Here's how the part is built. I have some questions about the finished solid (model axes, mm). A direction names the side the tool comes from. Give positions to 0.01 mm unless a question says otherwise; leave off trailing zeros. Loops run counter-clockwise (first coordinate to the right, second up) from the corner with the lowest first, then second, coordinate; pieces in that order, holes last. Notation, with made-up numbers: (70.5, 6.25) - (92.5, 6.25) arc R14 cw to (92.5, 24.25) - close; hole circle Ø8 at (-32, 35.25). An arc over 180 degrees is marked (long way). Use a Markdown table: item, result.
from build123d import *

# Parameters (mm, degrees)
SKETCH_1_W             = 43
SKETCH_1_H             = 44
EXTRUDE_1_DEPTH        = 17.5
SKETCH_2_W             = 50
SKETCH_2_H             = 68
CUT_EXTRUDE_1_DEPTH    = 52.373631369
HOLE_WIZARD_M4_1_D     = 3.3
HOLE_WIZARD_M4_1_DEPTH = 15.5
HOLE_WIZARD_M4_1_TIP   = 0.991420021
CHAMFER_1_SIZE         = 5
HOLE_WIZARD_M4_2_D     = 3.3
HOLE_WIZARD_M4_2_DEPTH = 15.5
HOLE_WIZARD_M4_2_TIP   = 0.991420021


with BuildPart() as part:
    # 草图1 → 凸台-拉伸1 (new, symmetric)
    with BuildSketch(Plane.XY):
        Rectangle(SKETCH_1_W, SKETCH_1_H)
    extrude(amount=EXTRUDE_1_DEPTH, both=True)

    # 草图2 → 切除-拉伸1 (cut, through all)
    with BuildSketch(Plane(origin=(21.5, 0, 0), x_dir=(0, 0, -1), z_dir=(1, 0, 0))):
        with Locations((17.5, -22)):
            Rectangle(SKETCH_2_W, SKETCH_2_H)
    extrude(amount=-CUT_EXTRUDE_1_DEPTH, mode=Mode.SUBTRACT)

    # M4 螺纹孔1
    with Locations(Plane(origin=(0, 0, -17.5), x_dir=(-1, 0, 0), z_dir=(0, 0, -1))):
        with Locations((-15, 17), (15, 17)):
            Hole(HOLE_WIZARD_M4_1_D / 2, depth=HOLE_WIZARD_M4_1_DEPTH)
            with Locations((0, 0, -(HOLE_WIZARD_M4_1_DEPTH + HOLE_WIZARD_M4_1_TIP / 2))):  # 118° drill point
                Cone(0, HOLE_WIZARD_M4_1_D / 2, HOLE_WIZARD_M4_1_TIP, mode=Mode.SUBTRACT)

    # 倒角1
    chamfer_1_edges = [part.edges().sort_by_distance(p)[0] for p in [
        (0, 22, 17.5),
    ]]
    chamfer(chamfer_1_edges, length=CHAMFER_1_SIZE)

    # M4 螺纹孔2
    with Locations(Plane(origin=(0, -22, 0), x_dir=(-1, 0, 0), z_dir=(0, -1, 0))):
        with Locations((10, -12.5), (-10, -12.5)):
            Hole(HOLE_WIZARD_M4_2_D / 2, depth=HOLE_WIZARD_M4_2_DEPTH)
            with Locations((0, 0, -(HOLE_WIZARD_M4_2_DEPTH + HOLE_WIZARD_M4_2_TIP / 2))):  # 118° drill point
                Cone(0, HOLE_WIZARD_M4_2_D / 2, HOLE_WIZARD_M4_2_TIP, mode=Mode.SUBTRACT)


solid = part.part
(1) Suppose I cut it at A-A on x = -19. Write out the boundary of the cut face in (y, z).
A:
| item | result |
|---|---|
| outline | (-22, 7.5) - (12, 7.5) - (12, -17.5) - (22, -17.5) - (22, 12.5) - (17, 17.5) - (-22, 17.5) - close |
(2) On a 3-axis mill with a long thin cutter (end or side, diameter ignored), from which of +Z, -Z, +X, -X, +Y, -Y can I reach the whole of each face in a straight line? I mean faces 4 (the face through (16.574, 17.496, -9.642)), 5 (the face through (21.5, 5, 8)), 6 (the face through (10.761, -14.142, 13.964)), 7 (the face through (0, 12, -5)). Say none if no direction works.
A:
| item | result |
|---|---|
| face 4 | -Z |
| face 5 | +Z, -Z, +X, +Y, -Y |
| face 6 | -Y |
| face 7 | -Z, +X, -X, -Y |
(3) Suppose I cut it at B-B on y = -11. Write out the boundary of the cut face in (x, z).
A:
| item | result |
|---|---|
| outline | (-21.5, 7.5) - (21.5, 7.5) - (21.5, 17.5) - (-21.5, 17.5) - close; hole circle Ø3.3 at (-10, 12.5); hole circle Ø3.3 at (10, 12.5) |
(4) If I drill on line 1 (X direction, y = 17, z = -5.5); line 2 (X direction, y = -10.25, z = 12.5); line 3 (Z direction, x = 10, y = -9.75), over which ranges is the centre line in solid material (lowest first)?
A:
| item | result |
|---|---|
| line 1 | -21.5 to -16.65, -13.35 to 13.35, 16.65 to 21.5 |
| line 2 | -21.5 to -11.65, -8.35 to 8.35, 11.65 to 21.5 |
| line 3 | 7.5 to 10.85, 14.15 to 17.5 |
(5) Suppose I cut it at C-C on y = -1.5. Write out the boundary of the cut face in (x, z).
A:
| item | result |
|---|---|
| outline | (-21.5, 7.5) - (21.5, 7.5) - (21.5, 17.5) - (-21.5, 17.5) - close |
(6) We'd pull the mould along X, two halves only. Please class faces 1 (the face through (0, 17, -17.5)), 2 (the face through (9.85, -5.68, 12.26)), 3 (the face through (-21.5, 5, 8)): pulls with the +X half, pulls with the -X half, needs draft (parallel to the pull), parting line crosses it, or undercut.
A:
| item | result |
|---|---|
| face 1 | needs draft |
| face 2 | undercut |
| face 3 | pulls with the -X half |
(7) Will these pins go through, and if not, where does the flat tip stop? pin 1 (4 mm diameter, centred on x = 12, z = -13.5, fed in from -Y); pin 2 (10 mm diameter, centred on x = 2.5, y = -7.5, fed in from -Z).
A:
| item | result |
|---|---|
| pin 1 | y = 12 |
| pin 2 | z = 7.5 |
